Can you work these out from the drawing? Everything is in mm from the part's minimum corner. A direction names the side the tool comes from. Coordinates: 2 decimals unless noted, no trailing zeros. Order: outer loops, then holes, each group sorted by start corner. A loop starts at its lowest first (then second) coordinate and runs counter-clockwise, first axis right, second up. Notation, with made-up numbers: (69.5, 26) -> (102.5, 26) arc R25 cw to (102.5, 42) -> close; hole circle Ø11 at (73, -8). An arc over 180 degrees is marked (long way). Write item = value, one per line. Start each with the question number.
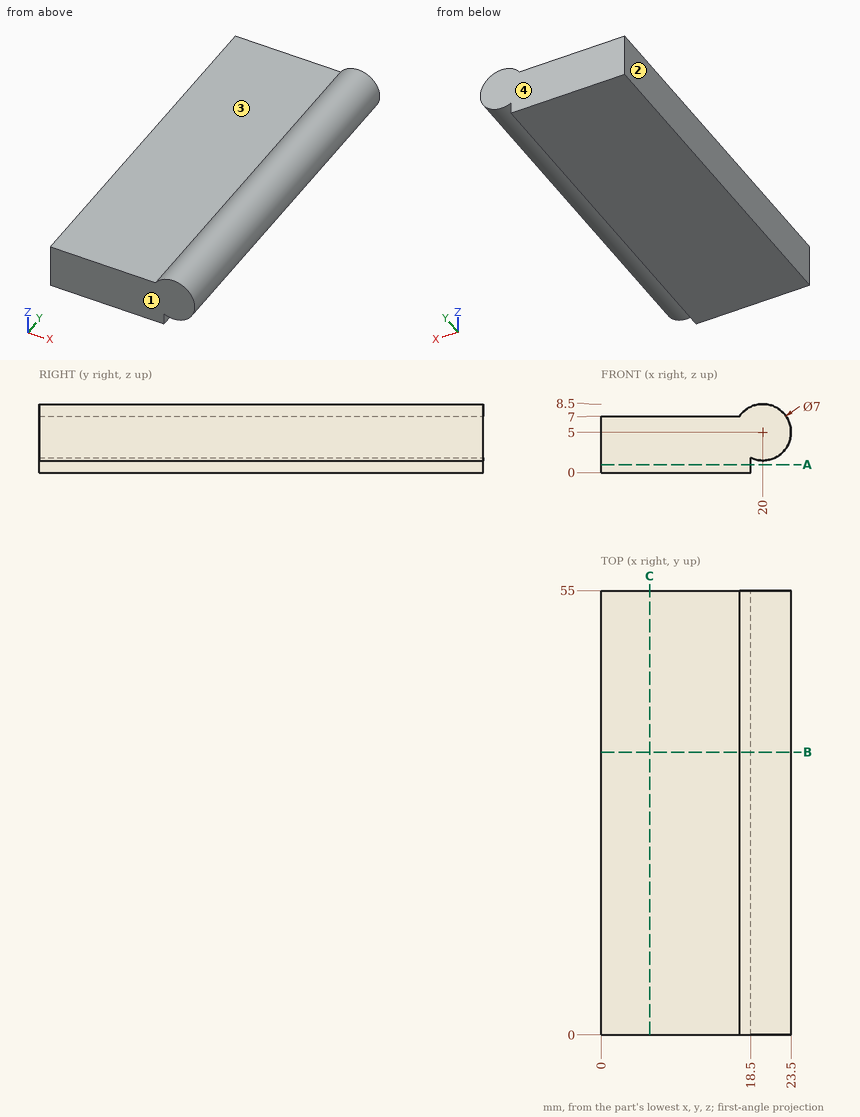
(1) For P1, Ø5, axis at x = 12, y = 33.5, coming from the +Z side; P2, Ø0.6, axis at y = 18, z = 1, coming from the +X side, each with a flat end and sliding along its axis, tell me the tip position at first contact or that it passes through.
(2) Imagine slicing it at B-B (y = 35). Write out the boundary of the cut face in (x, z).
(3) Imagine slicing it at A-A (z = 1). Write out the boundary of the cut face in (x, y).
(4) If I drill on L1, parallel to Z at x = 12, y = 6.5; L2, parallel to X at y = 39.5, z = 5.25; L3, parallel to X at y = 25, z = 6.25, over which ranges is the centre line in solid material (lowest first)? Write a range as from..to.
(5) For the marked faces 3 and 4, which set-ups out of +Z, -Z, +X, -X, +Y, -Y let a thin tool reach every point of the face, with its end or its side?
(6) Thinking about a two-plate mould opening in X: for the marked faces 1 and 2, which applies, +X half, -X half, draft (parallel to the pull), parting line (faces both ways), or undercut?
(7) Imagine slicing it at C-C (x = 6). Write out the boundary of the cut face in (y, z).
Result set:
q1.P1 = 7
q1.P2 = 18.5
q2.outline = (0, 0) -> (18.5, 0) -> (18.5, 1.84) arc R3.5 ccw (long way) to (17.13, 7) -> (0, 7) -> close
q3.outline = (0, 0) -> (18.5, 0) -> (18.5, 55) -> (0, 55) -> close
q4.L1 = 0..7
q4.L2 = 0..23.49
q4.L3 = 0..23.27
q5.face_3 = +Z, -X, +Y, -Y
q5.face_4 = +Z, -Z, +X, -X, +Y
q6.face_1 = draft
q6.face_2 = -X half
q7.outline = (0, 0) -> (55, 0) -> (55, 7) -> (0, 7) -> close
